```python
from build123d import *

# Parameters (mm, degrees)
SKETCH_1_R                   = 48
EXTRUDE_1_DEPTH              = 13
HOLE_WIZARD_M8_1_D           = 9
HOLE_WIZARD_M8_1_CBORE_D     = 14
HOLE_WIZARD_M8_1_CBORE_DEPTH = 8.6
SKETCH_3_R                   = 30
EXTRUDE_2_DEPTH              = 138
SKETCH_4_R                   = 20
CUT_EXTRUDE_3_DEPTH          = 166.556636835


with BuildPart() as part:
    # 草图1 → 拉伸1 (new body)
    with BuildSketch(Plane.XY):
        with Locations(Location((0, 0, 0), (0, 0, 180))):
            Circle(SKETCH_1_R)
    extrude(amount=EXTRUDE_1_DEPTH)

    # M8 六角凹头螺钉的柱形沉头孔1 (through all)
    with Locations(Plane(origin=(0, 39, 0), x_dir=(-1, 0, 0), z_dir=(0, 0, -1))):
        with Locations((0, 0), (-39, -39), (0, -78), (39, -39)):
            CounterBoreHole(HOLE_WIZARD_M8_1_D / 2, HOLE_WIZARD_M8_1_CBORE_D / 2, HOLE_WIZARD_M8_1_CBORE_DEPTH)

    # 草图3 → 拉伸2 (add)
    with BuildSketch(Plane.XY.offset(13)):
        Circle(SKETCH_3_R)
    extrude(amount=EXTRUDE_2_DEPTH)

    # 草图4 → 拉伸3 (cut, through all)
    with BuildSketch(Plane.XY.offset(151)):
        Circle(SKETCH_4_R)
    extrude(amount=-CUT_EXTRUDE_3_DEPTH, mode=Mode.SUBTRACT)


solid = part.part
```
Read the model definition and answer for the solid it produces. Units are mm, in the model's axes. A direction names the side the tool comes from. Coordinates: 2 decimals unless noted, no trailing zeros. Write each loop counter-clockwise with the first axis right and the second up, starting at its lowest first coordinate (ties: lowest second). Pieces come first, ordered by that corner, then holes. Notation, with made-up numbers: (77.5, 34.25) - (123.5, 34.25) arc R26 ccw to (123.5, 67.25) - close; hole circle Ø9 at (-23, 8). An arc over 180 degrees is marked (long way). Answer as a JSON object with one key per item and string values. Group by question number.
1. Which of the six approach directions +Z, -Z, +X, -X, +Y, -Y give full straight-line access (tool end or side, diameter ignored) to faces 4 (the flat face through (39, -5, 8.6)), 5 (the flat face through (-21, -22, 13)), 6 (the cylindrical face through (-0.98, 34.61, 10.83))?
2. The mould has two halves that part along X. Classify faces 1 (the cylindrical face through (-29.97, 1.32, 81.03)), 2 (the flat face through (-21, -1, 0)), 3 (the flat face through (-5, -39, 8.6)): +X half, -X half, draft (parallel to the pull), parting line (faces both ways), or undercut.
3. A cutting plane is placed at A-A (y = 0). Determine the outline of the cut face in (x, z), plus the area to 3 significant figures.
4. Each of these flat-tipped pins is pushed along its axis until it touches: P1, Ø1, axis at y = 11.5, z = 30.5, coming from the -X side; P2, Ø4, axis at x = -15.5, z = 21, coming from the +Y side; P3, Ø5, axis at x = -4.5, z = 116.5, coming from the -Y side. Where does it stop, or does it pass through?
5. Consider L1, parallel to Y at x = 0, z = 11; L2, parallel to Y at x = 0, z = 3; L3, parallel to Z at x = -33.5, y = -5.5. Determine where each line is inside the solid, lowest interval first. Write a range as [from, to].
6. A cutting plane is placed at C-C (y = 39). Determine the outline of the cut face in (x, z), plus the area to 3 significant figures.
Worked out:
{
 "1": {"face 4": "-Z", "face 5": "+Z", "face 6": "+Z, -Z"},
 "2": {"face 1": "parting line", "face 2": "draft", "face 3": "undercut"},
 "3": {"outline": "(-48, 0) - (-46, 0) - (-46, 8.6) - (-43.5, 8.6) - (-43.5, 13) - (-48, 13) - close; (-34.5, 8.6) - (-32, 8.6) - (-32, 0) - (-20, 0) - (-20, 151) - (-30, 151) - (-30, 13) - (-34.5, 13) - close; (20, 0) - (32, 0) - (32, 8.6) - (34.5, 8.6) - (34.5, 13) - (30, 13) - (30, 151) - (20, 151) - close; (43.5, 8.6) - (46, 8.6) - (46, 0) - (48, 0) - (48, 13) - (43.5, 13) - close", "area": "3,170 mm²"},
 "4": {"P1": "stops at x = -27.91", "P2": "stops at y = 26.79", "P3": "stops at y = -29.93"},
 "5": {"L1": "y = [-48, -43.5], [-34.5, -20], [20, 34.5], [43.5, 48]", "L2": "y = [-48, -46], [-32, -20], [20, 32], [46, 48]", "L3": "z = [0, 13]"},
 "6": {"outline": "(-27.98, 0) - (-7, 0) - (-7, 8.6) - (-4.5, 8.6) - (-4.5, 13) - (-27.98, 13) - close; (4.5, 8.6) - (7, 8.6) - (7, 0) - (27.98, 0) - (27.98, 13) - (4.5, 13) - close", "area": "568 mm²"}
}
